Source: CAD feature listing. Evaluate the final solid. Frame: model axes, mm. Face numbers are marked on the shaded views. A direction names the side the tool comes from. Give positions to 0.01 mm unless a question says otherwise; leave off trailing zeros. Loops run counter-clockwise (first coordinate to the right, second up) from the corner with the lowest first, then second, coordinate; pieces in that order, holes last.
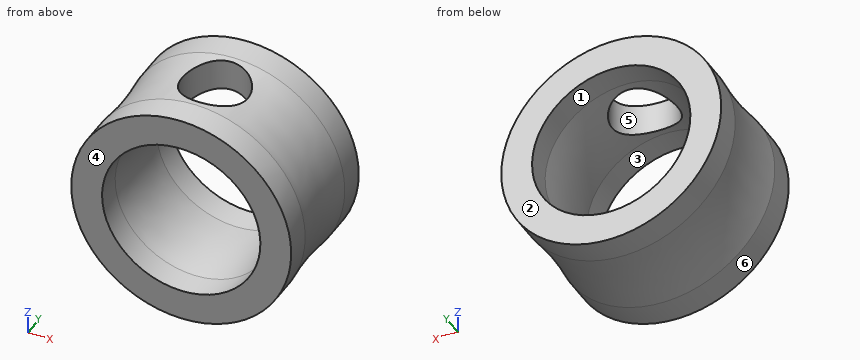
from build123d import *

# Parameters (mm, degrees)
SHELL1_T           = -70
SKETCH2_R          = 75
CUT_EXTRUDE1_DEPTH = 689


with BuildPart() as part:
    # Sketch1 → Revolve1 (revolve)
    with BuildSketch(Plane.XY, mode=Mode.PRIVATE) as revolve1_sk:
        with BuildLine():
            Line((0, 0), (0, 300))
            Line((0, 300), (250, 300))
            Line((250, 300), (250, 237.890484124))
            ThreePointArc((250, 237.890484124), (244.867735294, 150), (250, 62.109515876))
            Line((250, 62.109515876), (250, 0))
            Line((250, 0), (0, 0))
        make_face()
    revolve(revolve1_sk.sketch.rotate(Axis((0, 0, 0), (0, 1, 0)), 90), axis=Axis((0, 0, 0), (0, 1, 0)))

    # Shell1
    shell1_openings = [part.faces().sort_by_distance(p)[0] for p in [
        (0, 300, 0),
        (0, 0, 0),
    ]]
    offset(amount=SHELL1_T, openings=shell1_openings, kind=Kind.INTERSECTION)

    # Sketch2 → Cut-Extrude1 (cut)
    with BuildSketch(Plane.XY):
        with Locations(Location((0, 150, 0), (0, 0, 222.553028983))):
            Circle(SKETCH2_R)
    extrude(amount=CUT_EXTRUDE1_DEPTH, mode=Mode.SUBTRACT)


solid = part.part
1) Ray query, probe 1 along X at (y, z) = (281, 0); probe 2 along Z at (x, y) = (82, 134); probe 3 along X at (y, z) = (181, 0). Return the intervals inside material, ascending.
Checks:
probe 1: x = -250 to -180, 180 to 250
probe 2: z = -230.91 to -154.63, 154.63 to 230.91
probe 3: x = -245.5 to -175.45, 175.45 to 245.5
2) Pull-direction query (Y, two-part tool) for the marked faces 4, 5 and 6; classes: released by +Y, released by -Y, zero draft, split by the parting line, or undercut.
Checks:
face 4: released by -Y
face 5: undercut
face 6: zero draft
3) Cut plane A-A (z = 0). Return loops of the section in (x, y).
Checks:
outline: (-250, 0) - (-180, 0) - (-180, 58.11) arc R825.13 ccw to (-180, 241.89) - (-180, 300) - (-250, 300) - (-250, 237.89) arc R755.13 cw to (-250, 62.11) - close; (180, 0) - (250, 0) - (250, 62.11) arc R755.13 cw to (250, 237.89) - (250, 300) - (180, 300) - (180, 241.89) arc R825.13 ccw to (180, 58.11) - close
4) Reachability of the marked faces 1, 2 and 3 from +Z, -Z, +X, -X, +Y, -Y: full face, straight path, thin tool, end or side. Return the list, or none.
Checks:
face 1: +Y
face 2: +Z, -Z, +X, -X, +Y
face 3: -Y
5) Cut plane C-C (y = 150). Return loops of the section in (x, z).
Checks:
outline: (-75, 157.97) - (-75, 233.1) arc R244.87 ccw (long way) to (75, 233.1) - (75, 157.97) arc R174.87 cw (long way) to start
6) Cut plane B-B (x = 0). Return loops of the section in (y, z), and give its area (3 significant figures).
Checks:
outline: (0, -250) - (62.11, -250) arc R755.13 cw to (237.89, -250) - (300, -250) - (300, -180) - (241.89, -180) arc R825.13 ccw to (58.11, -180) - (0, -180) - close; (0, 180) - (58.11, 180) arc R825.13 ccw to (75, 178.28) - (75, 248.6) arc R755.13 cw to (62.11, 250) - (0, 250) - close; (225, 178.28) arc R825.13 ccw to (241.89, 180) - (300, 180) - (300, 250) - (237.89, 250) arc R755.13 cw to (225, 248.6) - close
area: 31,500 mm2
7) Contact query for flat-ended pins moving along their axis: P1, Ø2, axis at x = -42.5, y = 54.5, coming from the +Z side; P2, Ø12, axis at y = 128.5, z = -116.5, coming from the +X side; P3, Ø2, axis at x = -129, y = 183, coming from the -Z side. Output: stop coordinate, or through.
Checks:
P1: stops at z = 246.53
P2: stops at x = 218.87
P3: stops at z = -209.6
8) Cut plane D-D (x = 58). State how many separate pieces and enclosed holes the cut face has, and give its area (3 significant figures).
Checks:
separate pieces: 3
enclosed holes: 0
area: 36,800 mm2
